Verification items for the finished model (mm, model axes). A direction names the side the tool comes from. Give positions to 0.01 mm unless a question says otherwise; leave off trailing zeros. Order: outer loops, then holes, each group sorted by start corner. A loop starts at its lowest first (then second) coordinate and runs counter-clockwise, first axis right, second up.
(1) Access from +Z, -Z, +X, -X, +Y, -Y to the whole of each face (thin tool, end or side, straight path). Record for faces 1 (the face through (0, 0, 0)), 2 (the face through (-6, 0, -12)), 3 (the face through (-20, 0, -34)).
(2) Sectioned sample at A-A on y = 0. Record the cut outline in (x, z), plus the area to 3 significant figures.
(3) Scan lines: L1, parallel to Z at x = -23.5, y = 0.25; L2, parallel to Z at x = -27.5, y = 4; L3, parallel to X at y = -1.5, z = -136. Record each from-to range of solid material in increasing order.
(4) Sectioned sample at B-B on z = -91. Record the cut outline in (x, y).
(5) Gauge pin test, flat ends, axial feed: pin 1 (12 mm diameter, centred on x = -22, z = -131.5, fed in from +Y); pin 2 (5 mm diameter, centred on x = -19.5, z = -47, fed in from -Y); pin 3 (6 mm diameter, centred on y = -1, z = -82, fed in from -X); pin 4 (6 mm diameter, centred on y = -2.5, z = -32.5, fed in from +X). Record the tip position at first contact, or that the pin passes through.
(6) Mould release check, pull along Z, two halves, no side actions. Record for faces 4 (the face through (-20, 0, -126)), 5 (the face through (-46, 0, -80)), 6 (the face through (-6, 0, -148)), 7 (the face through (0, 0, -160)): pulls with the +Z half, pulls with the -Z half, needs draft (parallel to the pull), parting line crosses it, or undercut.
```python
from build123d import *

# Parameters (mm, degrees)
SKETCH2_R = 6


with BuildPart() as part:
    # Sweep1: sweep along a path in Sketch1
    with BuildLine(Plane(origin=(0, 0, 0), x_dir=(1, 0, 0), z_dir=(0, 1, 0))) as sweep1_path:
        Line((0, 160), (0, 136))
        ThreePointArc((0, 136), (-4.686291501, 124.686291501), (-16, 120))
        Line((-16, 120), (-24, 120))
        ThreePointArc((-24, 120), (-35.313708499, 115.313708499), (-40, 104))
        Line((-40, 104), (-40, 56))
        ThreePointArc((-40, 56), (-35.313708499, 44.686291501), (-24, 40))
        Line((-24, 40), (-16, 40))
        ThreePointArc((-16, 40), (-4.686291501, 35.313708499), (0, 24))
        Line((0, 24), (0, 0))
    # Sketch2 → Sweep1 (sweep)
    with BuildSketch(Plane.XY):
        Circle(SKETCH2_R)
    sweep(path=sweep1_path.line)


solid = part.part
```
Ans:
1. face 1: +Z, +X, -X, +Y, -Y
1. face 2: +Z
1. face 3: none
2. outline: (-46, -104) arc R22 ccw to (-24, -126) - (-16, -126) arc R10 cw to (-6, -136) - (-6, -160) - (6, -160) - (6, -136) arc R22 ccw to (-16, -114) - (-24, -114) arc R10 cw to (-34, -104) - (-34, -56) arc R10 cw to (-24, -46) - (-16, -46) arc R22 ccw to (6, -24) - (6, 0) - (-6, 0) - (-6, -24) arc R10 cw to (-16, -34) - (-24, -34) arc R22 ccw to (-46, -56) - close
2. area: 2,550 mm2
3. L1: z = -125.99 to -114.01, -45.99 to -34.01
3. L2: z = -124.17 to -114.98, -45.02 to -35.83
3. L3: x = -5.81 to 5.81
4. outline: circle Ø12 at (-40, 0)
5. pin 1: stops at y = 2.4
5. pin 2: stops at y = -3.97
5. pin 3: stops at x = -46
5. pin 4: stops at x = 5.11
6. face 4: undercut
6. face 5: undercut
6. face 6: needs draft
6. face 7: pulls with the -Z half
